Here's how the part is built. I have some questions about the finished solid (model axes, mm). Face numbers are marked on the shaded views. A direction names the side the tool comes from. Give positions to 0.01 mm unless a question says otherwise; leave off trailing zeros. Order: outer loops, then holes, each group sorted by start corner. A loop starts at its lowest first (then second) coordinate and runs counter-clockwise, first axis right, second up. Notation, with made-up numbers: M 21.5,-13.5 L 26.5,-13.5 A28 cw 26.5,22.5 Z; hole C -26,-12.5 d5. An arc over 180 degrees is marked long. Use one line per item in the form item = value.
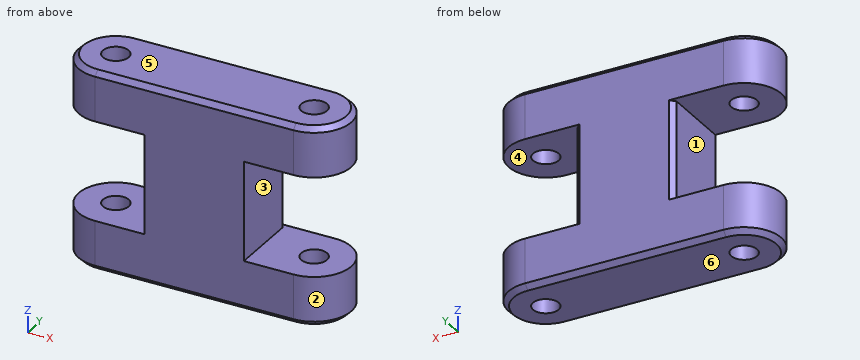
from build123d import *

# Parameters (mm, degrees)
SKETCH1_R           = 2.6
BOSS_EXTRUDE1_DEPTH = 5
SKETCH2_W           = 20
SKETCH2_H           = 15
BOSS_EXTRUDE2_DEPTH = 20
SKETCH3_R           = 2.6
BOSS_EXTRUDE3_DEPTH = 10
CHAMFER1_SIZE       = 1


with BuildPart() as part:
    # Sketch1 → Boss-Extrude1 (new, symmetric)
    with BuildSketch(Plane.XY):
        with BuildLine():
            Line((0, -7.5), (-40, -7.5))
            ThreePointArc((-40, -7.5), (-47.5, 0), (-40, 7.5))
            Line((-40, 7.5), (0, 7.5))
            ThreePointArc((0, 7.5), (7.5, 0), (0, -7.5))
        make_face()
        Circle(SKETCH1_R, mode=Mode.SUBTRACT)
        with Locations((-40, 0)):
            Circle(SKETCH1_R, mode=Mode.SUBTRACT)
    extrude(amount=BOSS_EXTRUDE1_DEPTH, both=True)

    # Sketch2 → Boss-Extrude2 (add)
    with BuildSketch(Plane(origin=(0, 0, -5), x_dir=(-1, 0, 0), z_dir=(0, 0, -1))):
        with Locations((20, 0)):
            Rectangle(SKETCH2_W, SKETCH2_H)
    extrude(amount=BOSS_EXTRUDE2_DEPTH)

    # Sketch3 → Boss-Extrude3 (add)
    with BuildSketch(Plane(origin=(0, 0, -25), x_dir=(-1, 0, 0), z_dir=(0, 0, -1))):
        with BuildLine():
            Line((0, 7.5), (40, 7.5))
            ThreePointArc((40, 7.5), (47.5, 0), (40, -7.5))
            Line((40, -7.5), (0, -7.5))
            ThreePointArc((0, -7.5), (-7.5, 0), (0, 7.5))
        make_face()
        with Locations(Location((0, 0, 0), (0, 0, 180))):
            Circle(SKETCH3_R, mode=Mode.SUBTRACT)
        with Locations(Location((40, 0, 0), (0, 0, 180))):
            Circle(SKETCH3_R, mode=Mode.SUBTRACT)
    extrude(amount=BOSS_EXTRUDE3_DEPTH)

    # Chamfer1
    chamfer1_edges = [part.edges().sort_by_distance(p)[0] for p in [
        (-47.5, 0, 5),
        (-20, -7.5, 5),
        (-30, 7.5, -15),
        (-10, 7.5, -15),
        (7.5, 0, -35),
        (-20, -7.5, -35),
        (-47.5, 0, -35),
        (-20, 7.5, -35),
        (7.5, 0, 5),
        (-20, 7.5, 5),
    ]]
    chamfer(chamfer1_edges, length=CHAMFER1_SIZE)


solid = part.part
Q1. I want a section at A-A on x = -1. Write out the boundary of the cut face in (y, z).
Found:
outline = M -7.5,-34 L -6.5,-35 L -2.4,-35 L -2.4,-25 L -7.5,-25 Z; M -7.5,-5 L -2.4,-5 L -2.4,5 L -6.5,5 L -7.5,4 Z; M 2.4,-35 L 6.5,-35 L 7.5,-34 L 7.5,-25 L 2.4,-25 Z; M 2.4,-5 L 7.5,-5 L 7.5,4 L 6.5,5 L 2.4,5 Z
Q2. I want a section at B-B on z = 0. Write out the boundary of the cut face in (x, y), then the cut area to 3 significant figures.
Found:
outline = M -40,-7.5 L 0,-7.5 A7.5 ccw 0,7.5 L -40,7.5 A7.5 ccw Z; hole C -40,0 d5.2; hole C 0,0 d5.2
area = 734 mm²
Q3. I'm going to push flat-ended pins straight in: pin 1 Ø8.5 at (x, y) = (-40, 0) entering from +Z; pin 2 Ø6 at (y, z) = (-5, -11) entering from +X; pin 3 Ø3 at (y, z) = (-5.5, -8) entering from -X; pin 4 Ø3 at (x, y) = (-40, 0) entering from +Z. Where does each tip first touch, or does it pass through?
Found:
pin_1 = 5
pin_2 = -10
pin_3 = -30
pin_4 = through
Q4. I want a section at C-C on z = -9. Write out the boundary of the cut face in (x, y), then the cut area to 3 significant figures.
Found:
outline = M -30,-7.5 L -10,-7.5 L -10,6.5 L -11,7.5 L -29,7.5 L -30,6.5 Z
area = 299 mm²
Q5. On a 3-axis mill with a long thin cutter (end or side, diameter ignored), from which of +Z, -Z, +X, -X, +Y, -Y can I reach the whole of each face in a straight line? I mean the marked faces 1 and 2. Say none if no direction works.
Found:
face_1 = -X, +Y, -Y
face_2 = +Z, -Z, +X
Q6. I want a section at D-D on y = 1. State how many separate pieces and enclosed holes the cut face has, then the cut area to 3 significant figures.
Found:
separate_pieces = 5
enclosed_holes = 0
area = 1,300 mm²
Q7. I need wall thicknesses on L1, parallel to Y at x = -40, z = 0; L2, parallel to Z at x = -3.5, y = -6.25; L3, parallel to X at y = 2.75, z = -18.5. Which ranges of each line are inside material? Lowest first, please.
Found:
L1 = -7.5 to -2.6, 2.6 to 7.5
L2 = -35 to -25, -5 to 5
L3 = -30 to -10
Q8. Thinking about a two-plate mould opening in Z: for the marked faces 3, 4, 5 and 6, which applies, +Z half, -Z half, draft (parallel to the pull), parting line (faces both ways), or undercut?
Found:
face_3 = undercut
face_4 = undercut
face_5 = +Z half
face_6 = -Z half
